Source: CAD feature listing. Evaluate the final solid. Frame: model axes, mm. Face numbers are marked on the shaded views. A direction names the side the tool comes from. Coordinates: 2 decimals unless noted, no trailing zeros. Loops run counter-clockwise (first coordinate to the right, second up) from the corner with the lowest first, then second, coordinate; pieces in that order, holes last. Notation, with made-up numbers: (59.25, 50) -> (115.25, 50) arc R19 cw to (115.25, 75) -> close; hole circle Ø3 at (-32.5, -35). An arc over 180 degrees is marked (long way). Answer as a JSON object with one key per item and string values. Group by question number.
from build123d import *

# Parameters (mm, degrees)
SKETCH2_R           = 34.5
SKETCH2_R_2         = 33.5
SKETCH2_R_3         = 30.5
SKETCH2_R_4         = 29.5
BOSS_EXTRUDE1_DEPTH = 5


with BuildPart() as part:
    # Sketch1 → Revolve1 (revolve)
    with BuildSketch(Plane.XY):
        Polygon((107, 42), (107, 35), (104.508470742, 35), (104.508470742, 27.05), (95.571275451, 27.05), (95.571275451, 21.43258158), (98.286326817, 21.43258158), (98.286326817, 24.55), (108, 24.55), (108, 31.426003585), (109.954236571, 31.426003585), (109.954236571, 42), align=None)
    revolve(axis=Axis((0, 0, 0), (-1, 0, 0)))

    # Sketch2 → Boss-Extrude1 (add)
    # profile 1 of 2: a face of its own
    with BuildSketch(Plane.ZY.offset(-104.508470742)):
        with Locations(Location((0, 0, 0), (0, 0, 270))):
            Circle(SKETCH2_R)
        with Locations(Location((0, 0, 0), (0, 0, 270))):
            Circle(SKETCH2_R_2, mode=Mode.SUBTRACT)
    # profile 2 of 2: a face of its own
    with BuildSketch(Plane.ZY.offset(-104.508470742)):
        with Locations(Location((0, 0, 0), (0, 0, 270))):
            Circle(SKETCH2_R_3)
        with Locations(Location((0, 0, 0), (0, 0, 270))):
            Circle(SKETCH2_R_4, mode=Mode.SUBTRACT)
    extrude(amount=BOSS_EXTRUDE1_DEPTH)


solid = part.part
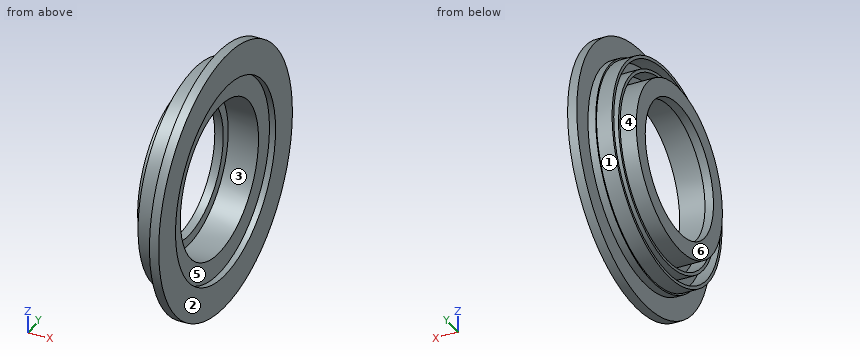
1. Section query B-B on x = 97. Return loops of the section in (y, z), then the cut area to 3 significant figures.
2. Pin query (flat end, axial travel): pin 1 Ø8 at (x, z) = (108.5, -32) entering from +Y; pin 2 Ø4 at (x, y) = (104.5, 19.5) entering from +Z; pin 3 Ø6 at (y, z) = (22.5, -24.5) entering from -X. Return the tip coordinate at first contact, or that it passes through.
3. Ray query, L1, parallel to Y at x = 109.5, z = 0; L2, parallel to Y at x = 97.6, z = 0; L3, parallel to Z at x = 100.9, y = 0. Return the intervals inside material, ascending.
4. Section query A-A on x = 102.5. Return loops of the section in (y, z), then the cut area to 3 significant figures.
5. Reachability of the marked faces 4, 5 and 6 from +Z, -Z, +X, -X, +Y, -Y: full face, straight path, thin tool, end or side. Return the list, or none.
6. Mould query, pull axis Y, two halves, no side actions, for the marked faces 1, 2 and 3. Classes: pulls with the +Y half, pulls with the -Y half, needs draft (parallel to the pull), parting line crosses it, or undercut.
Solved:
{
 "1": {"outline": "circle Ø54.1 at (0, 0); hole circle Ø42.87 at (0, 0)", "area": "856 mm^2"},
 "2": {"pin 1": "y = 31.3", "pin 2": "z = 30.31", "pin 3": "x = 99.51"},
 "3": {"L1": "-42 to -31.43, 31.43 to 42", "L2": "-27.05 to -21.43, 21.43 to 27.05", "L3": "-34.5 to -33.5, -30.5 to -29.5, -27.05 to -24.55, 24.55 to 27.05, 29.5 to 30.5, 33.5 to 34.5"},
 "4": {"outline": "circle Ø69 at (0, 0); circle Ø61 at (0, 0); circle Ø54.1 at (0, 0); hole circle Ø67 at (0, 0); hole circle Ø59 at (0, 0); hole circle Ø49.1 at (0, 0)", "area": "807 mm^2"},
 "5": {"face 4": "-X", "face 5": "+X", "face 6": "+Z, -Z, -X, +Y, -Y"},
 "6": {"face 1": "parting line crosses it", "face 2": "needs draft", "face 3": "undercut"}
}
